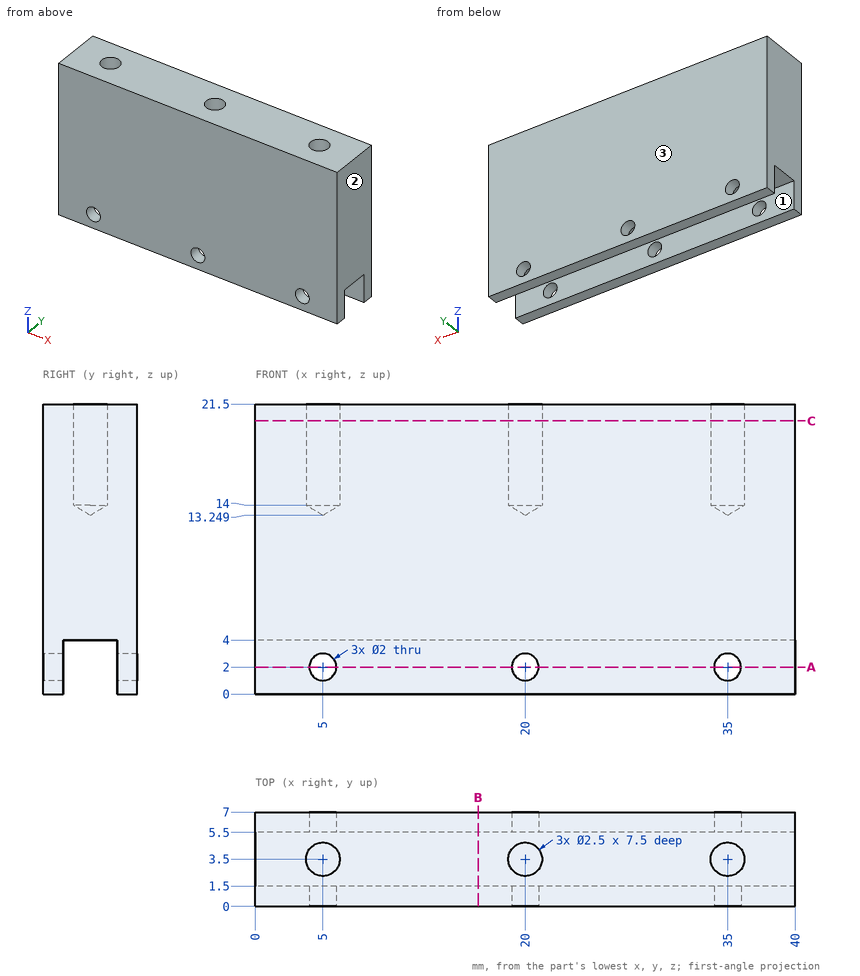
Study the drawing (mm; zero at the part's minimum x, y, z) and answer. Coordinates: 2 decimals unless noted, no trailing zeros. Write each loop counter-clockwise with the first axis right and the second up, starting at its lowest first coordinate (ties: lowest second). Pieces come first, ordered by that corner, then holes. Notation, with made-up numbers: (26, 57.25) - (48, 57.25) arc R26 ccw to (48, 82.25) - close; hole circle Ø7 at (12.5, 60.5). An arc over 180 degrees is marked (long way). Return JSON: item names as keys, results as strings. Group by question number.
1. A cutting plane is placed at A-A, the plane z = 2. Give the number of separate pieces and of enclosed holes in the cut face, plus the area to 3 significant figures.
2. Straight lines are drawn through the part: L1, parallel to X at y = 3.5, z = 18.25; L2, parallel to Z at x = 20, y = 6; L3, parallel to Y at x = 35, z = 18.5. For each, find the intervals that lie inside material, in ascending order.
3. A cutting plane is placed at C-C, the plane z = 20.25. Determine the outline of the cut face in (x, y).
4. A cutting plane is placed at B-B, the plane x = 16.5. Determine the outline of the cut face in (y, z), plus the area to 4 significant figures.
5. Given pin 1 (1.6 mm diameter, centred on x = 20, z = 2, fed in from +Y); pin 2 (1.5 mm diameter, centred on x = 35, y = 3.5, fed in from +Z); pin 3 (2 mm diameter, centred on x = 5, y = 3.5, fed in from -Z), each flat-ended and moving along its own axis, determine where each tip first touches the part or whether it passes through.
6. Determine the mould class of the marked faces 1, 2 and 3 for opening direction Y: released by +Y, released by -Y, zero draft, split by the parting line, or undercut.
Ans:
{
 "1": {"separate pieces": "8", "enclosed holes": "0", "area": "102 mm²"},
 "2": {"L1": "0 to 3.75, 6.25 to 18.75, 21.25 to 33.75, 36.25 to 40", "L2": "0 to 1, 3 to 21.5", "L3": "0 to 2.25, 4.75 to 7"},
 "3": {"outline": "(0, 0) - (40, 0) - (40, 7) - (0, 7) - close; hole circle Ø2.5 at (5, 3.5); hole circle Ø2.5 at (20, 3.5); hole circle Ø2.5 at (35, 3.5)"},
 "4": {"outline": "(0, 0) - (1.5, 0) - (1.5, 4) - (5.5, 4) - (5.5, 0) - (7, 0) - (7, 21.5) - (0, 21.5) - close", "area": "134.5 mm²"},
 "5": {"pin 1": "through", "pin 2": "z = 13.7", "pin 3": "z = 4"},
 "6": {"face 1": "undercut", "face 2": "zero draft", "face 3": "released by +Y"}
}
